Check sheet for the drawn part. Datum: minimum x, y, z corner. Units: mm. A direction names the side the tool comes from. Coordinates: 2 decimals unless noted, no trailing zeros. Loops run counter-clockwise (first coordinate to the right, second up) from the corner with the lowest first, then second, coordinate; pieces in that order, holes last. Notation, with made-up numbers: (-20.5, 85) -> (30.5, 85) arc R29 cw to (30.5, 108) -> close; hole circle Ø3 at (-11.5, 40). An arc over 180 degrees is marked (long way). Use CSV: the item, a comma, the result in double quotes. Start each with the question number.
1. Sectioned sample at A-A, the plane y = 24. Record the cut outline in (x, z), and give its area (3 significant figures).
2. Release check for a two-part mould opening along Y. For the marked faces 6, 7 and 8 record: pulls with the +Y half, pulls with the -Y half, needs draft (parallel to the pull), parting line crosses it, or undercut.
3. Set-up check for the marked faces 1, 2, 3, 4 and 5: record each of +Z, -Z, +X, -X, +Y, -Y from which the full face is reachable in a straight line by a thin tool's end or side.
4. Thickness scan on L1, parallel to Y at x = 33, z = 13; L2, parallel to Y at x = 107, z = 30.5; L3, parallel to X at y = 6, z = 13.5. Record the ranges inside material, lowest first.
5. Gauge pin test, flat ends, axial feed: pin 1 (12 mm diameter, centred on x = 51, y = 32, fed in from -Z); pin 2 (2.5 mm diameter, centred on x = 146.75, y = 35.25, fed in from -Z); pin 3 (1 mm diameter, centred on y = 42.5, z = 33.5, fed in from -X). Record the tip position at first contact, or that the pin passes through.
6. Sectioned sample at C-C, the plane z = 9. Record the cut outline in (x, y), and give its area (3 significant figures).
7. Sectioned sample at B-B, the plane x = 59.5. Record the cut outline in (y, z), and give its area (3 significant figures).
8. Sectioned sample at D-D, the plane y = 44. Record the cut outline in (x, z), and give its area (3 significant figures).
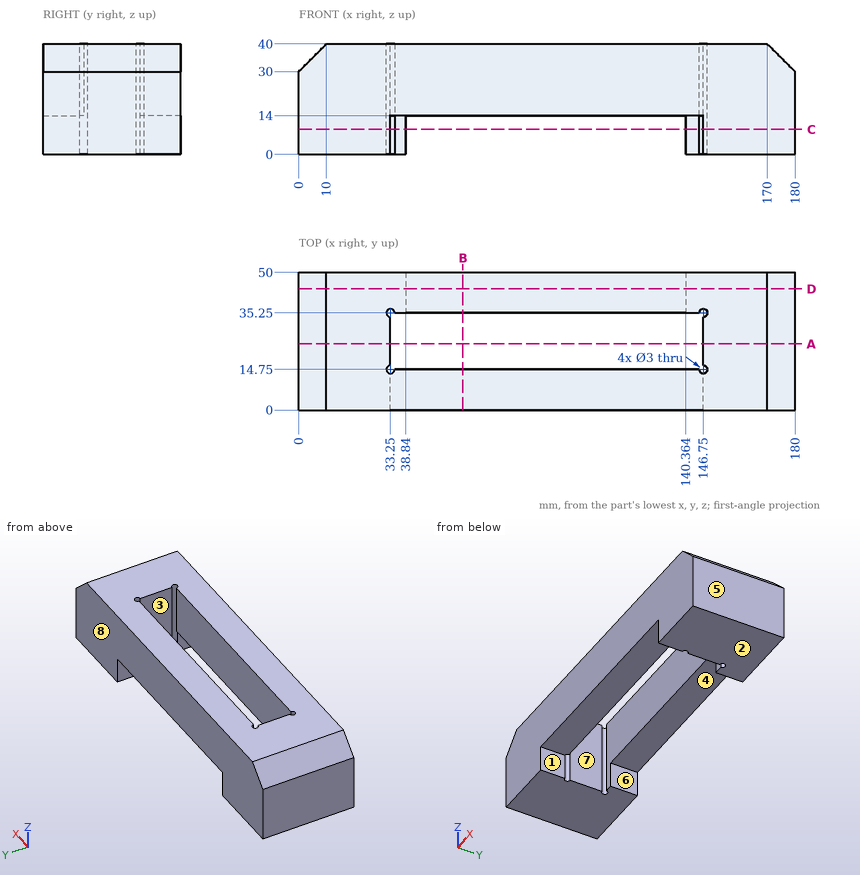
Completed:
1,outline,"(0, 0) -> (33.25, 0) -> (33.25, 40) -> (10, 40) -> (0, 30) -> close; (146.75, 0) -> (180, 0) -> (180, 30) -> (170, 40) -> (146.75, 40) -> close"
1,area,"2,560 mm²"
2,face 6,"needs draft"
2,face 7,"undercut"
2,face 8,"pulls with the +Y half"
3,face 1,"-Z, -Y"
3,face 2,"-Z, +X, -X, +Y, -Y"
3,face 3,"+Z, -Z"
3,face 4,"-Z, +Y, -Y"
3,face 5,"+Z, -Z, +X, +Y, -Y"
4,L1,"0 to 13.27, 16.23 to 33.77, 36.73 to 50"
4,L2,"0 to 14.75, 35.25 to 50"
4,L3,"0 to 33.25, 146.75 to 180"
5,pin 1,"z = 14"
5,pin 2,"through"
5,pin 3,"x = 3"
6,outline,"(0, 0) -> (33.25, 0) -> (33.25, 13.25) arc R1.5 cw to (33.25, 16.25) -> (33.25, 33.75) arc R1.5 cw (long way) to (34.75, 35.25) -> (38.84, 35.25) -> (38.84, 50) -> (0, 50) -> close; (140.36, 35.25) -> (145.25, 35.25) arc R1.5 cw (long way) to (146.75, 33.75) -> (146.75, 16.25) arc R1.5 cw to (146.75, 13.25) -> (146.75, 0) -> (180, 0) -> (180, 50) -> (140.36, 50) -> close"
6,area,"3,480 mm²"
7,outline,"(0, 14) -> (14.75, 14) -> (14.75, 40) -> (0, 40) -> close; (35.25, 14) -> (50, 14) -> (50, 40) -> (35.25, 40) -> close"
7,area,"767 mm²"
8,outline,"(0, 0) -> (38.84, 0) -> (38.84, 14) -> (140.36, 14) -> (140.36, 0) -> (180, 0) -> (180, 30) -> (170, 40) -> (10, 40) -> (0, 30) -> close"
8,area,"5,680 mm²"
